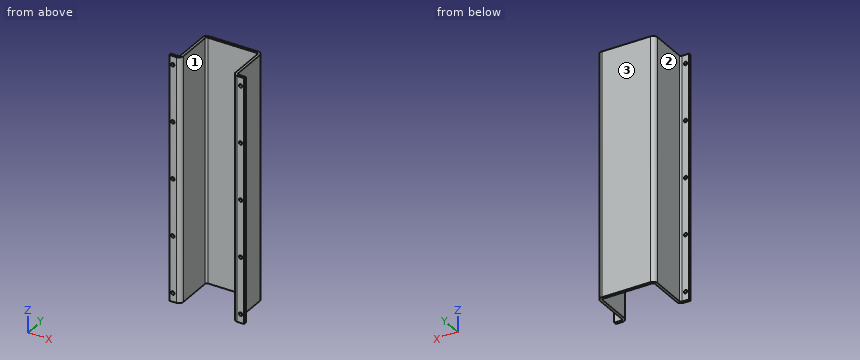
from build123d import *

# Parameters (mm, degrees)
BOSS_EXTRUDE1_DEPTH = 280
SKETCH7_R           = 2
CUT_EXTRUDE3_DEPTH  = 10
LPATTERN1_COUNT     = 5
LPATTERN1_PITCH     = 65


with BuildPart() as part:
    # Sketch1 → Boss-Extrude1 (new body)
    with BuildSketch(Plane.XY):
        with BuildLine():
            Line((86, 0), (86, 3))
            Line((86, 3), (78, 3))
            ThreePointArc((78, 3), (76.585786438, 3.585786438), (76, 5))
            Line((76, 5), (76, 46))
            ThreePointArc((76, 46), (74.535533906, 49.535533906), (71, 51))
            Line((71, 51), (15, 51))
            ThreePointArc((15, 51), (11.464466094, 49.535533906), (10, 46))
            Line((10, 46), (10, 5))
            ThreePointArc((10, 5), (9.414213562, 3.585786438), (8, 3))
            Line((8, 3), (0, 3))
            Line((0, 3), (0, 0))
            Line((0, 0), (8, 0))
            ThreePointArc((8, 0), (11.535533906, 1.464466094), (13, 5))
            Line((13, 5), (13, 46))
            ThreePointArc((13, 46), (13.585786438, 47.414213562), (15, 48))
            Line((15, 48), (71, 48))
            ThreePointArc((71, 48), (72.414213562, 47.414213562), (73, 46))
            Line((73, 46), (73, 5))
            ThreePointArc((73, 5), (74.464466094, 1.464466094), (78, 0))
            Line((78, 0), (86, 0))
        make_face()
    extrude(amount=BOSS_EXTRUDE1_DEPTH)

    # Sketch7 → Cut-Extrude3 (cut)
    with BuildSketch(Plane(origin=(0, 0, 0), x_dir=(-1, 0, 0), z_dir=(0, -1, 0))):
        with Locations(Location((-4, -270, 0), (0, 0, 180))):
            Circle(SKETCH7_R)
        with Locations(Location((-82, -270, 0), (0, 0, 180))):
            Circle(SKETCH7_R)
    cut_extrude3 = extrude(amount=-CUT_EXTRUDE3_DEPTH, mode=Mode.SUBTRACT)

    # LPattern1: Cut-Extrude3 ×5
    with Locations(*[(0, 0, -i * LPATTERN1_PITCH) for i in range(1, LPATTERN1_COUNT)]):
        add(cut_extrude3, mode=Mode.SUBTRACT)


solid = part.part
Part model, mm, in its own coordinate system. Face numbers are marked on the shaded views. A direction names the side the tool comes from. Coordinates: 2 decimals unless noted, no trailing zeros. Loops run counter-clockwise (first coordinate to the right, second up) from the corner with the lowest first, then second, coordinate; pieces in that order, holes last. Notation, with made-up numbers: (83.5, -16) - (102.5, -16) arc R24 cw to (102.5, -5) - close; hole circle Ø9 at (-40, 67). An arc over 180 degrees is marked (long way). Write each question's results on one line, items separated by ' | '. Start each with the question number.
Q1. Slice it at A-A on y = 32. Give the cut face in (x, z).
Q2. Which spindle directions (+Z, -Z, +X, -X, +Y, -Y) get a long thin tool onto all of the face, cutting with end or side? Do the marked faces 1, 2 and 3. Say none if no direction does.
Q3. Probe line 1 along Z through (x, y) = (82, 1); line 2 along X through (y, z) = (13.5, 212.5); line 3 along X through (y, z) = (1, 140). List the from-to ranges inside material, lowest first.
Q4. Slice it at C-C on x = 56.5. Give the cut face in (y, z).
Q5. Drop flat-ended pins along their axis: pin 1 Ø4.5 at (x, z) = (4, 75) entering from -Y; pin 2 Ø2.5 at (x, z) = (4.5, 154) entering from +Y; pin 3 Ø12 at (y, z) = (31.5, 29) entering from +X; pin 4 Ø4 at (x, z) = (37.5, 76) entering from -Y. Give the stop position or say it passes through.
Q6. Slice it at B-B on z = 49. Give the cut face in (x, y).
Answer:
1) outline: (10, 0) - (13, 0) - (13, 280) - (10, 280) - close; (73, 0) - (76, 0) - (76, 280) - (73, 280) - close
2) face 1: +Z, -Z, -Y | face 2: +Z, -Z, -X, +Y | face 3: +Z, -Z, +X, -X, +Y
3) line 1: z = 0 to 8, 12 to 73, 77 to 138, 142 to 203, 207 to 268, 272 to 280 | line 2: x = 10 to 13, 73 to 76 | line 3: x = 0 to 2, 6 to 11, 75 to 80, 84 to 86
4) outline: (48, 0) - (51, 0) - (51, 280) - (48, 280) - close
5) pin 1: stops at y = 0 | pin 2: stops at y = 3 | pin 3: stops at x = 76 | pin 4: stops at y = 48
6) outline: (0, 0) - (8, 0) arc R5 ccw to (13, 5) - (13, 46) arc R2 cw to (15, 48) - (71, 48) arc R2 cw to (73, 46) - (73, 5) arc R5 ccw to (78, 0) - (86, 0) - (86, 3) - (78, 3) arc R2 cw to (76, 5) - (76, 46) arc R5 ccw to (71, 51) - (15, 51) arc R5 ccw to (10, 46) - (10, 5) arc R2 cw to (8, 3) - (0, 3) - close
